from build123d import *

# Parameters (mm, degrees)
FILLET1_R = 1.1
FILLET2_R = 1.1


with BuildPart() as part:
    # Sketch1 → Revolve1 (revolve)
    with BuildSketch(Plane.XY, mode=Mode.PRIVATE) as revolve1_sk:
        Polygon((0, 20), (18, 20), (18, 25.3), (17.17, 25.3), (17.17, 34.825), (18, 34.825), (18, 40), (0, 40), (0, 34.825), (0.83, 34.825), (0.83, 25.3), (0, 25.3), align=None)
    revolve(revolve1_sk.sketch.rotate(Axis((0, 0, 0), (1, 0, 0)), 90), axis=Axis((0, 0, 0), (1, 0, 0)))

    # Fillet1
    fillet1_edges = [part.edges().sort_by_distance(p)[0] for p in [
        (0, 0, -40),
        (18, 0, -40),
    ]]
    fillet(fillet1_edges, radius=FILLET1_R)

    # Fillet2
    fillet2_edges = [part.edges().sort_by_distance(p)[0] for p in [
        (18, 0, -20),
        (0, 0, -20),
    ]]
    fillet(fillet2_edges, radius=FILLET2_R)


solid = part.part
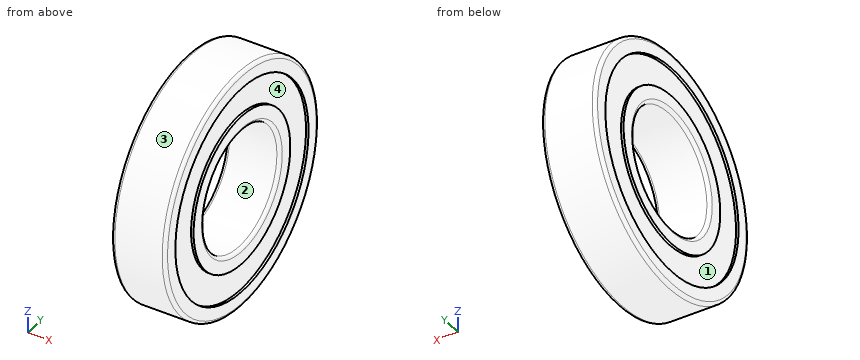
Read the model definition and answer for the solid it produces. Units are mm, in the model's axes. Face numbers are marked on the shaded views. A direction names the side the tool comes from. Coordinates: 2 decimals unless noted, no trailing zeros. Order: outer loops, then holes, each group sorted by start corner. A loop starts at its lowest first (then second) coordinate and runs counter-clockwise, first axis right, second up. Notation, with made-up numbers: M -9.75,73.25 L 46.25,73.25 A4 ccw 46.25,77.25 Z; hole C -9.5,36.5 d1. An arc over 180 degrees is marked long. Put each result on its own line as item: value. Start each with the question number.
Item 1: Section C-C, the plane x = 2.75 is taken. Determine the outline of the cut face in (y, z).
Item 2: For the marked faces 1 and 2, determine the directions among +Z, -Z, +X, -X, +Y, -Y from which every point of the face is accessible in a straight line to the end or side of a thin tool.
Item 3: Consider probe 1 along Y at (x, z) = (11.5, 0); probe 2 along Y at (x, z) = (17.55, 0) (3 decimals); probe 3 along X at (y, z) = (31.5, -13.5). Determine where each line is inside the solid, lowest interval first. Write a range as [from, to].
Item 4: Given pin 1 Ø2 at (y, z) = (-25.5, -9) entering from +X; pin 2 Ø3 at (x, y) = (2.5, -19) entering from -Z; pin 3 Ø2 at (x, y) = (5.5, 1) entering from -Z; pin 4 Ø1 at (x, z) = (14.5, -2.5) entering from -Y, each flat-ended and moving along its own axis, determine where each tip first touches the part or whether it passes through.
Item 5: The mould has two halves that part along Z. Classify the marked faces 3 and 4: +Z half, -Z half, draft (parallel to the pull), parting line (faces both ways), or undercut.
Computed:
1. outline: C 0,0 d80; hole C 0,0 d40
2. face 1: -X
2. face 2: +X, -X
3. probe 1: y = [-40, -20], [20, 40]
3. probe 2: y = [-39.787, -34.825], [-25.3, -20.213], [20.213, 25.3], [34.825, 39.787]
3. probe 3: x = [0.83, 17.17]
4. pin 1: stops at x = 17.17
4. pin 2: stops at z = -35.97
4. pin 3: stops at z = -40
4. pin 4: stops at y = -39.95
5. face 3: parting line
5. face 4: undercut
